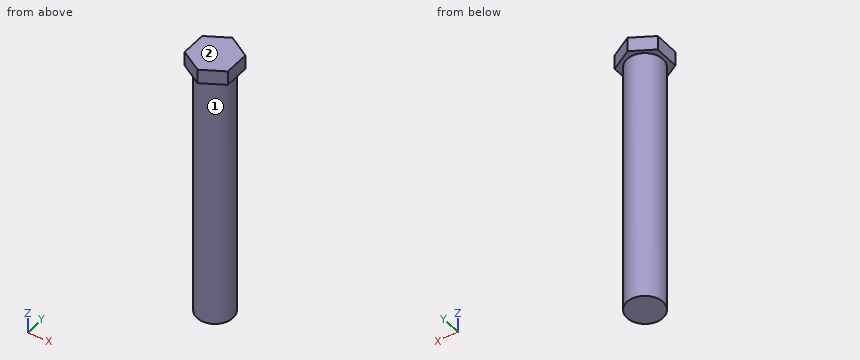
from build123d import *

# Parameters (mm, degrees)
SKETCH_1_R      = 5
EXTRUDE_1_DEPTH = 72
EXTRUDE_2_DEPTH = 4


with BuildPart() as part:
    # 草图1 → 凸台-拉伸1 (new body)
    with BuildSketch(Plane.XY):
        Circle(SKETCH_1_R)
    extrude(amount=EXTRUDE_1_DEPTH)

    # 草图2 → 凸台-拉伸2 (add)
    with BuildSketch(Plane.XY.offset(72)):
        Polygon((5.987217074, -3.486148549), (6.012701742, 3.44200781), (0.025484667, 6.928156359), (-5.987217074, 3.486148549), (-6.012701742, -3.44200781), (-0.025484667, -6.928156359), align=None)
    extrude(amount=EXTRUDE_2_DEPTH)


solid = part.part
Read the model definition and answer for the solid it produces. Units are mm, in the model's axes. Face numbers are marked on the shaded views. A direction names the side the tool comes from. Give positions to 0.01 mm unless a question says otherwise; leave off trailing zeros. Write each loop counter-clockwise with the first axis right and the second up, starting at its lowest first coordinate (ties: lowest second). Pieces come first, ordered by that corner, then holes. Notation, with made-up numbers: (-37.75, 87) - (-1.75, 87) arc R6 cw to (-1.75, 97) - close; hole circle Ø2 at (80, 3.25). An arc over 180 degrees is marked (long way). Use CSV: the item, a comma, the result in double quotes. Start each with the question number.
(1) Given P1, Ø5, axis at x = -0.5, z = 48, coming from the +Y side; P2, Ø1, axis at y = -3.5, z = 42.5, coming from the +X side; P3, Ø4, axis at x = 0, z = 36.5, coming from the -Y side, each flat-ended and moving along its own axis, determine where each tip first touches the part or whether it passes through.
(2) Find section A-A (x = -4.25). Give the vertices of the cut face in (y, z), plus the area to 3 significant figures.
(3) For the marked faces 1 and 2, determine the directions among +Z, -Z, +X, -X, +Y, -Y from which every point of the face is accessible in a straight line to the end or side of a thin tool.
(4) Find section C-C (y = 4.25). Give the vertices of the cut face in (x, z).
(5) Consider line 1 along Z through (x, y) = (-5.25, 3); line 2 along Y through (x, z) = (-0.25, 23.5); line 3 along Y through (x, z) = (1.75, 32). Determine where each line is inside the solid, lowest interval first.
(6) Find section B-B (z = 61.5). Give the vertices of the cut face in (x, y), plus the area to 3 significant figures.
Findings below:
1,P1,"y = 5"
1,P2,"x = 4"
1,P3,"y = -5"
2,outline,"(-4.47, 72) - (-2.63, 72) - (-2.63, 0) - (2.63, 0) - (2.63, 72) - (4.48, 72) - (4.48, 76) - (-4.47, 76) - close"
2,area,"415 mm2"
3,face 1,"-Z"
3,face 2,"+Z, +X, -X, +Y, -Y"
4,outline,"(-4.65, 72) - (-2.63, 72) - (-2.63, 0) - (2.63, 0) - (2.63, 72) - (4.63, 72) - (4.63, 76) - (-4.65, 76) - close"
5,line 1,"72 to 76"
5,line 2,"-4.99 to 4.99"
5,line 3,"-4.68 to 4.68"
6,outline,"circle Ø10 at (0, 0)"
6,area,"78.5 mm2"
